Source: three-view drawing plus pictorial views. Frame: mm from the lowest corner of the part. A direction names the side the tool comes from. Coordinates: 2 decimals unless noted, no trailing zeros. Write each loop counter-clockwise with the first axis right and the second up, starting at its lowest first coordinate (ties: lowest second). Pieces come first, ordered by that corner, then holes.
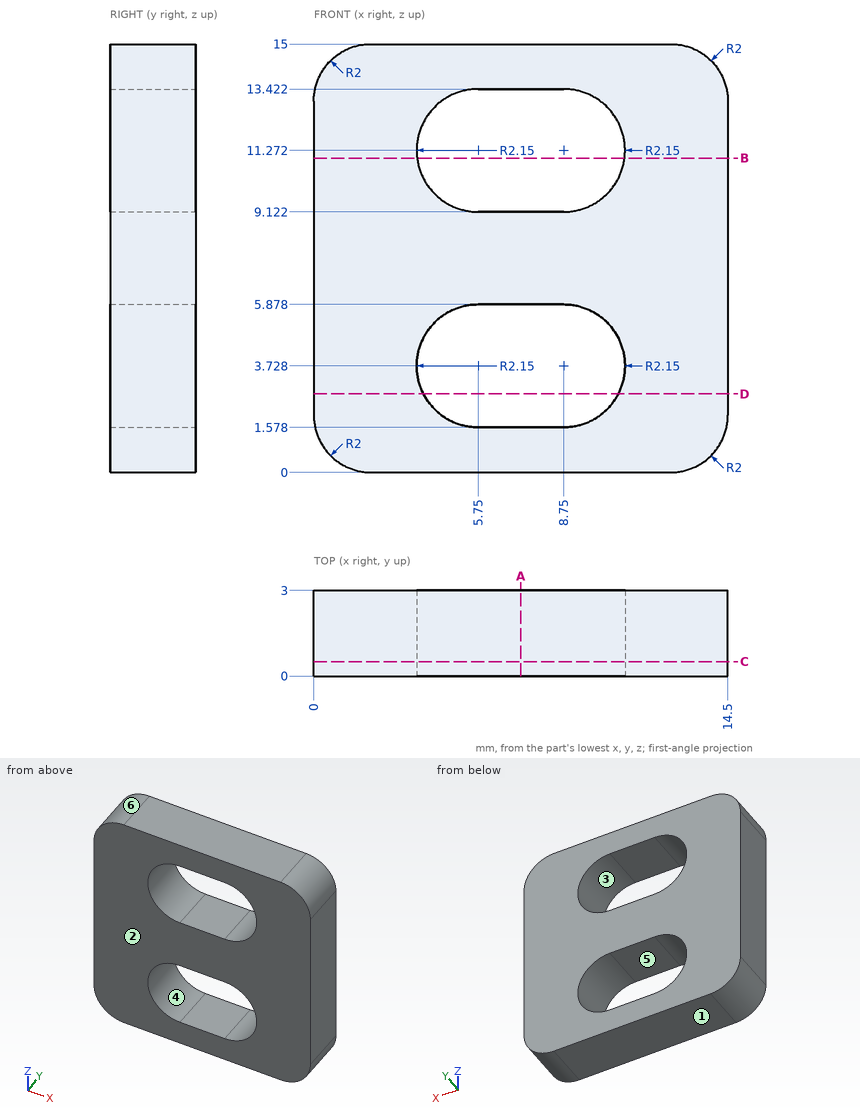
Item 1: Pull-direction query (Z, two-part tool) for the marked faces 1, 2, 3 and 4; classes: released by +Z, released by -Z, zero draft, split by the parting line, or undercut.
Item 2: Section query C-C, the plane y = 0.5. Return loops of the section in (x, z).
Item 3: Section query A-A, the plane x = 7.25. Return loops of the section in (y, z), then the cut area to 3 significant figures.
Item 4: Access query for the marked faces 5 and 6. Directions: +Z, -Z, +X, -X, +Y, -Y. A direction counts if a zero-diameter tool reaches every point of the face in a straight line with its end or side. Return the directions, or none.
Item 5: Section query B-B, the plane z = 11. Return loops of the section in (x, y).
Item 6: Section query D-D, the plane z = 2.75. Return loops of the section in (x, y) (1 decimal).
Item 7: Material intervals for line 1 (X direction, y = 1, z = 11.25); line 2 (Z direction, x = 8.25, y = 1.8); line 3 (Z direction, x = 9.5, y = 1.8), sorted ascending.
The answers:
1. face 1: released by -Z
1. face 2: zero draft
1. face 3: undercut
1. face 4: undercut
2. outline: (0, 2) arc R2 ccw to (2, 0) - (12.5, 0) arc R2 ccw to (14.5, 2) - (14.5, 13) arc R2 ccw to (12.5, 15) - (2, 15) arc R2 ccw to (0, 13) - close; hole (5.75, 1.58) - (8.75, 1.58) arc R2.15 ccw to (8.75, 5.88) - (5.75, 5.88) arc R2.15 ccw to start; hole (5.75, 9.12) - (8.75, 9.12) arc R2.15 ccw to (8.75, 13.42) - (5.75, 13.42) arc R2.15 ccw to start
3. outline: (0, 0) - (3, 0) - (3, 1.58) - (0, 1.58) - close; (0, 5.88) - (3, 5.88) - (3, 9.12) - (0, 9.12) - close; (0, 13.42) - (3, 13.42) - (3, 15) - (0, 15) - close
3. area: 19.2 mm2
4. face 5: +Y, -Y
4. face 6: +Z, -X, +Y, -Y
5. outline: (0, 0) - (3.62, 0) - (3.62, 3) - (0, 3) - close; (10.88, 0) - (14.5, 0) - (14.5, 3) - (10.88, 3) - close
6. outline: (0, 0) - (3.8, 0) - (3.8, 3) - (0, 3) - close; (10.7, 0) - (14.5, 0) - (14.5, 3) - (10.7, 3) - close
7. line 1: x = 0 to 3.6, 10.9 to 14.5
7. line 2: z = 0 to 1.58, 5.88 to 9.12, 13.42 to 15
7. line 3: z = 0 to 1.71, 5.74 to 9.26, 13.29 to 15
